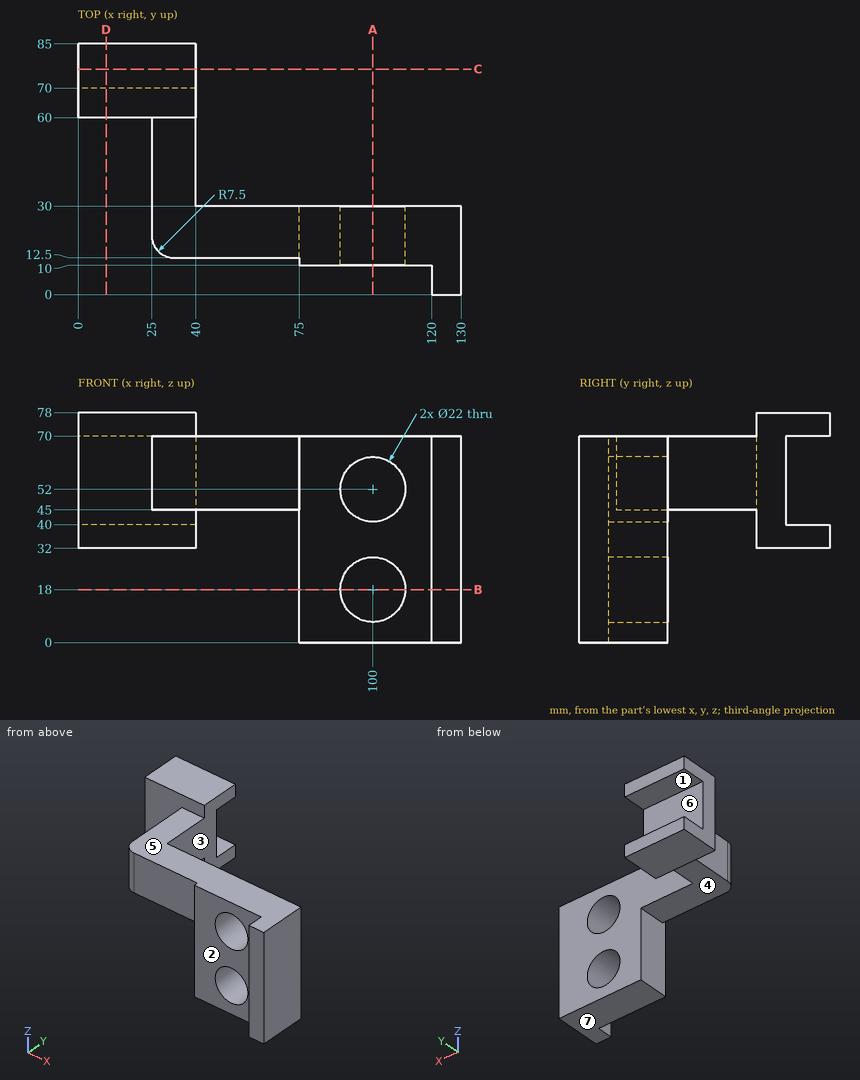
The figure shows three views and two pictorial views of one solid part (mm, origin at its lowest corner). Answer the questions. A direction names the side the tool comes from. Coordinates: 2 decimals unless noted, no trailing zeros. Write each loop counter-clockwise with the first axis right and the second up, starting at its lowest first coordinate (ties: lowest second). Pieces come first, ordered by that corner, then holes. Notation, with made-up numbers: M 49,15 L 91,15 A21 cw 91,46 Z; hole C 45.25,31.25 d7. An arc over 180 degrees is marked long. Answer as CSV lines item,"result". Start each with the question number.
Item 1: Section C-C on y = 76.5 is taken. Write down the section's boundary in (x, z), and give its area (3 significant figures).
Item 2: Consider L1, parallel to Z at x = 10, y = 74; L2, parallel to X at y = 11.5, z = 18.5; L3, parallel to Z at x = 66, y = 13. Determine where each line is inside the solid, lowest interval first.
Item 3: Flat-ended cylindrical pins translate along their axes: P1, Ø22.5, axis at x = 96, z = 33.5, coming from the -Y side; P2, Ø4.5, axis at x = 26, y = 74.5, coming from the -Z side; P3, Ø7.5, axis at y = 39, z = 54, coming from the -X side; P4, Ø10, axis at x = 100.5, z = 54.5, coming from the +Y side (3 decimals). Find the tip coordinate at first contact, or state that the pin passes through.
Item 4: A tool of negligible diameter and unlimited length cuts with its end or side. For the marked faces 1, 2, 3 and 4, from which of +Z, -Z, +X, -X, +Y, -Y can it reach the whole face along a straight path? Write none if from no direction.
Item 5: Section A-A on x = 100 is taken. Write down the section's boundary in (y, z).
Item 6: Section B-B on z = 18 is taken. Write down the section's boundary in (x, y).
Item 7: Determine the mould class of the marked faces 5, 6 and 7 for opening direction Z: released by +Z, released by -Z, zero draft, split by the parting line, or undercut.
Item 8: Section D-D on x = 9.5 is taken. Write down the section's boundary in (y, z).
Checks:
1,outline,"M 0,32 L 40,32 L 40,40 L 0,40 Z; M 0,70 L 40,70 L 40,78 L 0,78 Z"
1,area,"640 mm²"
2,L1,"z = 32 to 40, 70 to 78"
2,L2,"x = 75 to 89.01, 110.99 to 130"
2,L3,"z = 45 to 70"
3,P1,"stops at y = 10"
3,P2,"stops at z = 32"
3,P3,"stops at x = 25"
3,P4,"passes through"
4,face 1,"+X, -X, +Y"
4,face 2,"+Z, -Z, -X, -Y"
4,face 3,"+Z, -Z, +X, +Y"
4,face 4,"-Z, -X, -Y"
5,outline,"M 10,0 L 30,0 L 30,7 L 10,7 Z; M 10,29 L 30,29 L 30,41 L 10,41 Z; M 10,63 L 30,63 L 30,70 L 10,70 Z"
6,outline,"M 75,10 L 89,10 L 89,30 L 75,30 Z; M 111,10 L 120,10 L 120,0 L 130,0 L 130,30 L 111,30 Z"
7,face 5,"released by +Z"
7,face 6,"undercut"
7,face 7,"released by -Z"
8,outline,"M 60,32 L 85,32 L 85,40 L 70,40 L 70,70 L 85,70 L 85,78 L 60,78 Z"
